Build history of the part. All positions in model axes, mm. A direction names the side the tool comes from. Give positions to 0.01 mm unless a question says otherwise; leave off trailing zeros. Order: outer loops, then holes, each group sorted by start corner. A loop starts at its lowest first (then second) coordinate and runs counter-clockwise, first axis right, second up. Notation, with made-up numbers: M 48,5 L 87,5 A16 cw 87,21 Z; hole C 46.25,60.5 d7. An arc over 180 degrees is marked long. One line per item, written item: value. Start each with the question number.
from build123d import *

# Parameters (mm, degrees)
SKETCH2_R           = 2.5
BOSS_EXTRUDE1_DEPTH = 17.9
CUT_EXTRUDE1_DEPTH  = 3.95
SKETCH4_W           = 7.9
SKETCH4_H           = 17.88597718
CUT_EXTRUDE2_DEPTH  = 41.9
SKETCH5_R           = 6.2
CUT_EXTRUDE3_DEPTH  = 41.9


with BuildPart() as part:
    # Sketch2 → Boss-Extrude1 (new body)
    with BuildSketch(Plane.XY):
        with BuildLine():
            Line((5, -30.431019852), (5, 0))
            ThreePointArc((5, 0), (0, 5), (-5, 0))
            Line((-5, 0), (-5, -21.316065276))
            Line((-5, -21.316065276), (-28.5, -34.883796602))
            Line((-28.5, -34.883796602), (-28.5, -49.07456062))
            ThreePointArc((-28.5, -49.07456062), (-19.40948098, -53.327615248), (-9.711912859, -55.9128004))
            Line((-9.711912859, -55.9128004), (5, -30.431019852))
        make_face()
        with Locations(Location((0, 0, 0), (0, 0, 180))):
            Circle(SKETCH2_R, mode=Mode.SUBTRACT)
    extrude(amount=BOSS_EXTRUDE1_DEPTH)

    # Sketch3 → Cut-Extrude1 (cut, symmetric)
    with BuildSketch(Plane(origin=(0, 0, 8.95), x_dir=(-1, 0, 0), z_dir=(0, 0, -1))):
        Polygon((1.84861519, -9.72875797), (-2.55, -34.674544331), (-5, -30.431019852), (-5, -8.521162332), align=None)
    extrude(amount=CUT_EXTRUDE1_DEPTH, both=True, mode=Mode.SUBTRACT)

    # Sketch4 → Cut-Extrude2 (cut)
    with BuildSketch(Plane.ZY.offset(5)):
        with Locations((8.95, -1.613076686)):
            Rectangle(SKETCH4_W, SKETCH4_H)
    extrude(amount=-CUT_EXTRUDE2_DEPTH, mode=Mode.SUBTRACT)

    # Sketch5 → Cut-Extrude3 (cut)
    with BuildSketch(Plane(origin=(19.409643134, -53.32755623, 0), x_dir=(0, 0, -1), z_dir=(0.34202014332566744, -0.9396926207859089, 0))):
        with Locations((-8.95, -39.667670129)):
            Circle(SKETCH5_R)
    extrude(amount=-CUT_EXTRUDE3_DEPTH, mode=Mode.SUBTRACT)


solid = part.part
1) Drill centre lines: line 1 (Z direction, x = -25.5, y = -34.5); line 2 (Z direction, x = -1, y = -12); line 3 (Y direction, x = 0, z = 2.6). Where is each one in solid material? Low to high.
2) Slice it at B-B (z = 14.5). List the corners of the cut face in (x, y), plus the area to 3 significant figures.
3) Tool access for faces 1 (the flat face through (-3, -10.556, 9)), 2 (the flat face through (-2.46, -43.35, 8.82)), 3 (the flat face through (1, -11, 5)): list every direction of +Z, -Z, +X, -X, +Y, -Y with a clear straight run to the whole face (end or side of a thin tool).
4) Pull direction Y, two halves, no side cores. Call faces 4 (the cylindrical face through (2.5, -0.1, 15.4)), 5 (the cylindrical face through (0, 5, 2)), 6 (the flat face through (-5, -13, 9)), 7 (the cylindrical face through (2.5, -0.1, 2.5)): pulls with the +Y half, pulls with the -Y half, needs draft (parallel to the pull), parting line crosses it, or undercut.
5) Slice it at A-A (y = -4.5). List the corners of the cut face in (x, z).
6) Slice it at D-D (y = -22). List the corners of the cut face in (x, z), plus the area to 3 significant figures.
7) Slice it at C-C (x = 0). List the corners of the cut face in (y, z).
8) Drop flat-ended pins along their axis: P1, Ø3, axis at y = -41.5, z = 5, coming from the -X side; P2, Ø2, axis at y = -19, z = 6.5, coming from the -X side; P3, Ø5, axis at y = -22.5, z = 9, coming from the +X side; P4, Ø10, axis at y = -27, z = 12.5, coming from the +X side. Give the stop position or say it passes through.
Results list:
1. line 1: z = 0 to 4.13, 13.77 to 17.9
1. line 2: z = 0 to 5, 12.9 to 17.9
1. line 3: y = -39.09 to -2.5, 2.5 to 5
2. outline: M -28.5,-49.07 A56.75 ccw -26.98,-49.92 L -28.5,-45.76 Z; M -26.91,-33.97 L -19.93,-53.13 A56.75 ccw -9.71,-55.91 L 5,-30.43 L 5,0 A5 ccw -5,0 L -5,-21.32 Z; hole C 0,0 d5
2. area: 915 mm²
3. face 1: +X, -X, +Y
3. face 2: +Z, -Z, +X, -Y
3. face 3: +X, +Y
4. face 4: undercut
4. face 5: pulls with the +Y half
4. face 6: needs draft
4. face 7: undercut
5. outline: M -5,0 L 5,0 L 5,5 L -5,5 Z; M -5,12.9 L 5,12.9 L 5,17.9 L -5,17.9 Z
6. outline: M -6.18,0 L 5,0 L 5,5 L 0.32,5 L 0.32,12.9 L 5,12.9 L 5,17.9 L -6.18,17.9 Z
6. area: 163 mm²
7. outline: M -39.09,0 L -2.5,0 L -2.5,5 L -20.21,5 L -20.21,12.9 L -2.5,12.9 L -2.5,17.9 L -39.09,17.9 Z; M 2.5,0 L 5,0 L 5,5 L 2.5,5 Z; M 2.5,12.9 L 5,12.9 L 5,17.9 L 2.5,17.9 Z
8. P1: stops at x = -24.01
8. P2: stops at x = -5
8. P3: stops at x = 0.84
8. P4: stops at x = 5
